```python
from build123d import *

# Parameters (mm, degrees)
SKETCH1_R           = 8
BOSS_EXTRUDE1_DEPTH = 1.5


with BuildPart() as part:
    # Sketch1 → Boss-Extrude1 (new body)
    with BuildSketch(Plane.XZ.offset(1.5)):
        with Locations(Location((0, 0, 0), (0, 0, 90))):
            Circle(SKETCH1_R)
        with BuildLine():
            Line((3, 2.332380758), (3, -2.332380758))
            ThreePointArc((3, -2.332380758), (2.687005769, -2.687005769), (2.332380758, -3))
            Line((2.332380758, -3), (-2.332380758, -3))
            ThreePointArc((-2.332380758, -3), (-2.687005769, -2.687005769), (-3, -2.332380758))
            Line((-3, -2.332380758), (-3, 2.332380758))
            ThreePointArc((-3, 2.332380758), (-2.687005769, 2.687005769), (-2.332380758, 3))
            Line((-2.332380758, 3), (2.332380758, 3))
            ThreePointArc((2.332380758, 3), (2.687005769, 2.687005769), (3, 2.332380758))
        make_face(mode=Mode.SUBTRACT)
    extrude(amount=-BOSS_EXTRUDE1_DEPTH)


solid = part.part
```
Work out the finished part from the listing and answer in its coordinate system (mm). A direction names the side the tool comes from. Coordinates: 2 decimals unless noted, no trailing zeros. Loops run counter-clockwise (first coordinate to the right, second up) from the corner with the lowest first, then second, coordinate; pieces in that order, holes last.
1) A flat-ended cylindrical pin translates along its axis: pin 1 (4 mm diameter, centred on x = -2.5, z = -4.5, fed in from +Y). Find the tip coordinate at first contact, or state that the pin passes through.
Results:
pin 1: stops at y = 0
2) For a pull along Z with two mould halves and no side action, classify faces 3 (the cylindrical face through (7.81, -0.76, -1.73)), 4 (the flat face through (-0.1, -1.5, 3.4)), 5 (the flat face through (0, -1, 3)) as +Z half, -Z half, draft (parallel to the pull), parting line (faces both ways), or undercut.
Results:
face 3: parting line
face 4: draft
face 5: undercut
3) Section A-A (z = 0) is taken. Give the vertices of the cut face in (x, y), plus the area to 3 significant figures.
Results:
outline: (-8, -1.5) - (-3, -1.5) - (-3, 0) - (-8, 0) - close; (3, -1.5) - (8, -1.5) - (8, 0) - (3, 0) - close
area: 15.0 mm2
4) Section D-D (z = 6) is taken. Give the vertices of the cut face in (x, y), plus the area to 3 significant figures.
Results:
outline: (-5.29, -1.5) - (5.29, -1.5) - (5.29, 0) - (-5.29, 0) - close
area: 15.9 mm2
5) For faces 1 (the flat face through (3, -1, 0)), 2 (the flat face through (-0.1, 0, 3.4)), determine the directions among +Z, -Z, +X, -X, +Y, -Y from which every point of the face is accessible in a straight line to the end or side of a thin tool.
Results:
face 1: +Y, -Y
face 2: +Z, -Z, +X, -X, +Y
6) Consider probe 1 along X at (y, z) = (-0.45, -2.75); probe 2 along X at (y, z) = (-0.15, 1.25); probe 3 along Z at (x, y) = (-1.75, -0.95). Determine where each line is inside the solid, lowest interval first.
Results:
probe 1: x = -7.51 to -2.62, 2.62 to 7.51
probe 2: x = -7.9 to -3, 3 to 7.9
probe 3: z = -7.81 to -3, 3 to 7.81
7) Section B-B (y = -1.2) is taken. Give the vertices of the cut face in (x, z).
Results:
outline: circle Ø16 at (0, 0); hole (-3, -2.33) arc R3.8 ccw to (-2.33, -3) - (2.33, -3) arc R3.8 ccw to (3, -2.33) - (3, 2.33) arc R3.8 ccw to (2.33, 3) - (-2.33, 3) arc R3.8 ccw to (-3, 2.33) - close
8) Section C-C (x = 0) is taken. Give the vertices of the cut face in (y, z), plus the area to 3 significant figures.
Results:
outline: (-1.5, -8) - (0, -8) - (0, -3) - (-1.5, -3) - close; (-1.5, 3) - (0, 3) - (0, 8) - (-1.5, 8) - close
area: 15.0 mm2
